```python
from build123d import *

# Parameters (mm, degrees)
BASE_PROFILE_DEPTH      = 10
SIDE_BLOCK_SKETCH_W     = 50
SIDE_BLOCK_SKETCH_H     = 50
SIDE_BLOCK_DEPTH        = 10
WEB_DEPTH               = 10
GUSSET_DEPTH            = 10
RAIL_SKETCH_W           = 55
RAIL_SKETCH_H           = 60
RAIL_DEPTH              = 10
POCKET_CUT_DEPTH        = 10
RELIEF_CUT_DEPTH        = 10
ARM_MOUNT_DEPTH         = 10
HOOK_ARM_DEPTH          = 10
RING_BOSS_DEPTH         = 10
BORE_18_SKETCH_R        = 9
BORE_18_DEPTH           = 10
HOOK_CUTOUT_18_SKETCH_R = 9
HOOK_CUTOUT_18_DEPTH    = 10


with BuildPart() as part:
    # Base Profile Sketch → Base Profile (new body)
    with BuildSketch(Plane.XY):
        Polygon((0, 0), (125, 0), (125, 40), (125, 50), (80, 50), (80, 10), (0, 10), align=None)
    extrude(amount=BASE_PROFILE_DEPTH)

    # Side Block Sketch → Side Block (add)
    with BuildSketch(Plane(origin=(125, 0, 0), x_dir=(0, 0, -1), z_dir=(1, 0, 0))):
        with Locations((-35, 25)):
            Rectangle(SIDE_BLOCK_SKETCH_W, SIDE_BLOCK_SKETCH_H)
    extrude(amount=-SIDE_BLOCK_DEPTH)

    # Web Sketch → Web (add)
    with BuildSketch(Plane.XZ):
        Polygon((115, 60), (70, 60), (0, 40), (0, 10), (115, 10), align=None)
    extrude(amount=-WEB_DEPTH)

    # Gusset Sketch → Gusset (add)
    with BuildSketch(Plane(origin=(0, 0, 0), x_dir=(-1, 0, 0), z_dir=(0, 0, -1))):
        Polygon((-80, 50), (0, 10), (-80, 10), align=None)
    extrude(amount=-GUSSET_DEPTH)

    # Rail Sketch → Rail (add)
    with BuildSketch(Plane.XZ):
        with Locations((97.5, 30)):
            Rectangle(RAIL_SKETCH_W, RAIL_SKETCH_H)
    extrude(amount=RAIL_DEPTH)

    # Pocket Cut Sketch → Pocket Cut (cut)
    with BuildSketch(Plane.XY.offset(60)):
        Polygon((115, 50), (125, 50), (125, -10), (70, -10), (70, 10), (115, 10), align=None)
    extrude(amount=-POCKET_CUT_DEPTH, mode=Mode.SUBTRACT)

    # Relief Cut Sketch → Relief Cut (cut)
    with BuildSketch(Plane(origin=(0, 10, 0), x_dir=(1, 0, 0), z_dir=(0, 1, 0))):
        Polygon((0, -40), (0, -10), (70, -10), (70, -60), align=None)
    extrude(amount=-RELIEF_CUT_DEPTH, mode=Mode.SUBTRACT)

    # Arm Mount Sketch → Arm Mount (add)
    with BuildSketch(Plane(origin=(0, 10, 0), x_dir=(1, 0, 0), z_dir=(0, 1, 0))):
        Polygon((70, -10), (0, -10), (0, -26), (70, -50), align=None)
    extrude(amount=-ARM_MOUNT_DEPTH)

    # Hook Arm Sketch → Hook Arm (add)
    with BuildSketch(Plane.XZ):
        with BuildLine():
            Line((0, 0), (-19, 0))
            ThreePointArc((-19, 0), (-23.242640687, 1.757359313), (-25, 6))
            Line((-25, 6), (-25, 26))
            Line((-25, 26), (-19, 26))
            Line((-19, 26), (-18.5, 26))
            Line((-18.5, 26), (-18.5, 16))
            ThreePointArc((-18.5, 16), (-12.5, 10), (-6.5, 16))
            Line((-6.5, 16), (-6.5, 26))
            Line((-6.5, 26), (-6, 26))
            Line((-6, 26), (0, 26))
            Line((0, 26), (0, 0))
        make_face()
    extrude(amount=-HOOK_ARM_DEPTH)

    # Ring Boss Sketch → Ring Boss (add)
    with BuildSketch(Plane(origin=(125, 0, 0), x_dir=(0, 0, -1), z_dir=(1, 0, 0))):
        with BuildLine():
            Line((-50, 50), (-50, 18))
            ThreePointArc((-50, 18), (-66, 34), (-50, 50))
        make_face()
    extrude(amount=-RING_BOSS_DEPTH)

    # Bore Ø18 Sketch → Bore Ø18 (cut)
    with BuildSketch(Plane(origin=(125, 0, 0), x_dir=(0, 0, -1), z_dir=(1, 0, 0))):
        with Locations((-50, 34)):
            Circle(BORE_18_SKETCH_R)
    extrude(amount=-BORE_18_DEPTH, mode=Mode.SUBTRACT)

    # Hook Cutout Ø18 Sketch → Hook Cutout Ø18 (cut)
    with BuildSketch(Plane(origin=(0, 10, 0), x_dir=(1, 0, 0), z_dir=(0, 1, 0))):
        with Locations(Location((92.205854711, -25, 0), (0, 0, 270))):
            Circle(HOOK_CUTOUT_18_SKETCH_R)
    extrude(amount=-HOOK_CUTOUT_18_DEPTH, mode=Mode.SUBTRACT)


solid = part.part
```
For this review, take the finished solid that the model builds, in its own axes (mm). A direction names the side the tool comes from. Coordinates: 2 decimals unless noted, no trailing zeros. Write each loop counter-clockwise with the first axis right and the second up, starting at its lowest first coordinate (ties: lowest second). Pieces come first, ordered by that corner, then holes.
(1) Add section B-B on x = 113. Give the boundary of the cut face in (y, z).
(2) The part is to be moulded in two halves that separate along X. For faces 1 (the face through (-18.5, 5, 21)), 2 (the face through (70, 20, 0)), 3 (the face through (40.6, 30.3, 4.9)), say which applies: +X half, -X half, draft (parallel to the pull), parting line (faces both ways), or undercut.
(3) Tool access review of faces 4 (the face through (34, 0, 20)), 5 (the face through (84.22, 5.07, 29.15)), 6 (the face through (-22, 5, 26)), 7 (the face through (69, 26, 10)): name each direction out of +Z, -Z, +X, -X, +Y, -Y from which nothing blocks a thin tool from reaching the whole face with its end or side.
(4) For pin 1 Ø23.5 at (y, z) = (34, 50) entering from -X; pin 2 Ø3 at (x, y) = (-23, 5.5) entering from +Z; pin 3 Ø1 at (x, y) = (58, 19.5) entering from +Z, all flat-tipped, find the tip position at first contact; note any pin that passes through.
(5) Wall thickness on probe 1 along X at (y, z) = (8.25, 25); probe 2 along X at (y, z) = (-4, 44.5); probe 3 along Y at (x, z) = (43, 18.5): over which ranges is each line inside the solid? List them lowest first.
(6) Add section D-D on y = 6.5. Give the boundary of the cut face in (x, z).
(7) Add section A-A on y = 34. Give the boundary of the cut face in (x, z).
(8) Add section C-C on z = 21. Give the boundary of the cut face in (x, y).
Answer sheet:
1. outline: (-10, 0) - (50, 0) - (50, 10) - (10, 10) - (10, 50) - (-10, 50) - close
2. face 1: undercut
2. face 2: draft
2. face 3: -X half
3. face 4: +Z, -Z, -X, -Y
3. face 5: +Y
3. face 6: +Z, -X, +Y, -Y
3. face 7: +Z, -X, +Y
4. pin 1: stops at x = 115
4. pin 2: stops at z = 26
4. pin 3: stops at z = 10
5. probe 1: x = -25 to -18.5, -6.5 to 83.21, 101.21 to 125
5. probe 2: x = 70 to 125
5. probe 3: y = 0 to 10
6. outline: (-25, 6) arc R6 ccw to (-19, 0) - (125, 0) - (125, 50) - (70, 50) - (0, 26) - (-6.5, 26) - (-6.5, 16) arc R6 cw to (-18.5, 16) - (-18.5, 26) - (-25, 26) - close; hole circle Ø18 at (92.21, 25)
7. outline: (48, 0) - (125, 0) - (125, 41) - (115, 41) - (115, 10) - (48, 10) - close; (115, 59) - (125, 59) - (125, 66) - (115, 66) - close
8. outline: (-25, 0) - (-18.5, 0) - (-18.5, 10) - (-25, 10) - close; (-6.5, 0) - (70, 0) - (70, -10) - (125, -10) - (125, 50) - (115, 50) - (115, 10) - (100.27, 10) - (100.27, 0) - (84.14, 0) - (84.14, 10) - (-6.5, 10) - close
